Could you check a few things on this model? Use its own coordinates, in mm. A direction names the side the tool comes from. Round coordinates to 2 decimals unless told otherwise and drop trailing zeros. Loops run counter-clockwise (first coordinate to the right, second up) from the corner with the lowest first, then second, coordinate; pieces in that order, holes last. Notation, with made-up numbers: (16.5, 46.25) -> (67.5, 46.25) arc R29 ccw to (67.5, 74.25) -> close; hole circle Ø5 at (-27, -17). An arc over 180 degrees is marked (long way). One line per item, written item: value.
```python
from build123d import *

# Parameters (mm, degrees)
L_BODY_DEPTH               = 40
LUG_END_ROUND_RADIUS       = 20
LUG_END_ROUND_LENGTH       = 40
LUG_BORE_SKETCH_R          = 10
LUG_BORE_20_DEPTH          = 40
BASE_END_ROUND_RADIUS      = 20
BASE_END_ROUND_LENGTH      = 10
RING_BOSS_SKETCH_R         = 10
RING_BOSS_SKETCH_R_2       = 8
RING_BOSS_20X_16_DEPTH     = 5
INNER_CORNER_FILLET_R5_R   = 5
RING_BOSS_BASE_FILLET_R2_R = 2


with BuildPart() as part:
    # L Profile Sketch → L Body (new body)
    with BuildSketch(Plane.XY):
        Polygon((0, 0), (100, 0), (100, 10), (40, 10), (40, 40), (0, 40), align=None)
    extrude(amount=L_BODY_DEPTH)

    # Lug End Round: full round fillet: the end face becomes a half cylinder, R = half its width
    lug_end_round_face = Plane((0, 20, 20), x_dir=(0, 1, 0), z_dir=(-1, 0, 0))  # on the end face: x along it, z out of the body
    lug_end_round_slab = lug_end_round_face.offset(-LUG_END_ROUND_RADIUS / 2) * Box(LUG_END_ROUND_LENGTH, 2 * LUG_END_ROUND_RADIUS, LUG_END_ROUND_RADIUS, mode=Mode.PRIVATE)  # the body's end, R deep
    lug_end_round_round = Plane((20, 20, 20), x_dir=(-1, 0, 0), z_dir=(0, 1, 0)) * Cylinder(LUG_END_ROUND_RADIUS, LUG_END_ROUND_LENGTH, mode=Mode.PRIVATE)  # its axis R under the face
    add(lug_end_round_slab - lug_end_round_round, mode=Mode.SUBTRACT)

    # Lug Bore Sketch → Lug Bore _20 (cut)
    with BuildSketch(Plane(origin=(0, 40, 0), x_dir=(1, 0, 0), z_dir=(0, 1, 0))):
        with Locations(Location((20, -20, 0), (0, 0, 270))):
            Circle(LUG_BORE_SKETCH_R)
    extrude(amount=-LUG_BORE_20_DEPTH, mode=Mode.SUBTRACT)

    # Base End Round: full round fillet: the end face becomes a half cylinder, R = half its width
    base_end_round_face = Plane((100, 5, 20), x_dir=(0, -1, 0), z_dir=(1, 0, 0))  # on the end face: x along it, z out of the body
    base_end_round_slab = base_end_round_face.offset(-BASE_END_ROUND_RADIUS / 2) * Box(BASE_END_ROUND_LENGTH, 2 * BASE_END_ROUND_RADIUS, BASE_END_ROUND_RADIUS, mode=Mode.PRIVATE)  # the body's end, R deep
    base_end_round_round = Plane((80, 5, 20), x_dir=(1, 0, 0), z_dir=(0, -1, 0)) * Cylinder(BASE_END_ROUND_RADIUS, BASE_END_ROUND_LENGTH, mode=Mode.PRIVATE)  # its axis R under the face
    add(base_end_round_slab - base_end_round_round, mode=Mode.SUBTRACT)

    # Ring Boss Sketch → Ring Boss _20x_16 (add)
    with BuildSketch(Plane(origin=(0, 10, 0), x_dir=(1, 0, 0), z_dir=(0, 1, 0))):
        with Locations(Location((80, -20, 0), (0, 0, 90))):
            Circle(RING_BOSS_SKETCH_R)
        with Locations(Location((80, -20, 0), (0, 0, 270))):
            Circle(RING_BOSS_SKETCH_R_2, mode=Mode.SUBTRACT)
    extrude(amount=RING_BOSS_20X_16_DEPTH)

    # Inner Corner Fillet R5
    inner_corner_fillet_r5_edges = [part.edges().sort_by_distance(p)[0] for p in [
        (40, 10, 20),
    ]]
    fillet(inner_corner_fillet_r5_edges, radius=INNER_CORNER_FILLET_R5_R)

    # Ring Boss Base Fillet R2
    ring_boss_base_fillet_r2_edges = [part.edges().sort_by_distance(p)[0] for p in [
        (80, 10, 30),
    ]]
    fillet(ring_boss_base_fillet_r2_edges, radius=RING_BOSS_BASE_FILLET_R2_R)


solid = part.part
```
(1) Please list where these lines run through material, in increasing order: L1, parallel to X at y = 9, z = 20; L2, parallel to X at y = 16, z = 20; L3, parallel to X at y = 11.45, z = 20.
Results below:
L1: x = 0 to 10, 30 to 100
L2: x = 0 to 10, 30 to 40
L3: x = 0 to 10, 30 to 41.48, 69.92 to 72, 88 to 90.08
(2) We'd pull the mould along Z, two halves only. Please class faces 1 (the face through (29, 40, 15)), 2 (the face through (23, 20.28, 29.54)), 3 (the face through (36, 16, 40)): +Z half, -Z half, draft (parallel to the pull), parting line (faces both ways), or undercut.
Results below:
face 1: draft
face 2: undercut
face 3: +Z half
(3) Imagine slicing it at A-A on z = 20. Write out the boundary of the cut face in (x, y).
Results below:
outline: (0, 0) -> (10, 0) -> (10, 40) -> (0, 40) -> close; (30, 0) -> (100, 0) -> (100, 10) -> (92, 10) arc R2 cw to (90, 12) -> (90, 15) -> (88, 15) -> (88, 10) -> (72, 10) -> (72, 15) -> (70, 15) -> (70, 12) arc R2 cw to (68, 10) -> (45, 10) arc R5 cw to (40, 15) -> (40, 40) -> (30, 40) -> close
(4) For pin 1 Ø5 at (x, z) = (45, 16.5) entering from +Y; pin 2 Ø12.5 at (y, z) = (32, 12) entering from +X; pin 3 Ø16 at (x, z) = (78.5, 17.5) entering from +Y, each with a flat end and sliding along its axis, tell me the tip position at first contact or that it passes through.
Results below:
pin 1: stops at y = 10.67
pin 2: stops at x = 40
pin 3: stops at y = 15
(5) Imagine slicing it at B-B on y = 34.5. Write out the boundary of the cut face in (x, z), then the cut area to 3 significant figures.
Results below:
outline: (20, 0) -> (40, 0) -> (40, 40) -> (20, 40) arc R20 ccw to start; hole circle Ø20 at (20, 20)
area: 1,110 mm²
(6) On a 3-axis mill with a long thin cutter (end or side, diameter ignored), from which of +Z, -Z, +X, -X, +Y, -Y can I reach the whole of each face in a straight line? I mean faces 4 (the face through (67, 10, 20)), 5 (the face through (71.8, 15, 20)), 6 (the face through (41, 12, 20)). Say none if no direction works.
Results below:
face 4: +Y
face 5: +Z, -Z, +X, +Y
face 6: +Z, -Z, +Y
(7) Imagine slicing it at D-D on x = 54. Write out the boundary of the cut face in (y, z).
Results below:
outline: (0, 0) -> (10, 0) -> (10, 40) -> (0, 40) -> close
(8) Imagine slicing it at C-C on z = 4.5. Write out the boundary of the cut face in (x, y).
Results below:
outline: (7.36, 0) -> (92.64, 0) -> (92.64, 10) -> (45, 10) arc R5 cw to (40, 15) -> (40, 40) -> (7.36, 40) -> close
